Geometry check sheet. Reference: the model listing, model coordinates, mm. Face numbers are marked on the shaded views. A direction names the side the tool comes from. Coordinates: 2 decimals unless noted, no trailing zeros. Loops run counter-clockwise (first coordinate to the right, second up) from the corner with the lowest first, then second, coordinate; pieces in that order, holes last. Notation, with made-up numbers: (-4, 52.5) -> (7, 52.5) arc R13 cw to (7, 65.5) -> close; hole circle Ø4 at (86, -10). An arc over 180 degrees is marked (long way). Answer as a JSON object with one key per item and string values.
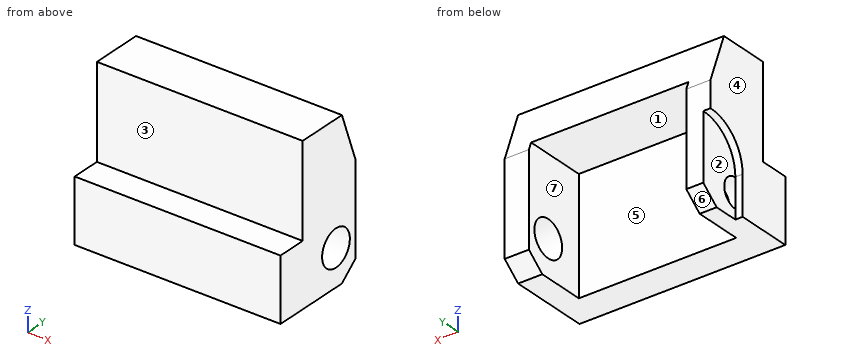
from build123d import *

# Parameters (mm, degrees)
BEARING_BLOCK_DEPTH    = 42.5
LUG_SLOT_PROFILE_W     = 65
LUG_SLOT_PROFILE_H     = 50
LUG_SLOT_65X50_DEPTH   = 27
BORE_15_SKETCH_R       = 7.5
PIVOT_BORE_15_DEPTH    = 10
LUG_RECESS_A_3MM_DEPTH = 3
LUG_RECESS_B_3MM_DEPTH = 3
BORE_10_SKETCH_R       = 6
PIVOT_BORE_10_DEPTH    = 7


with BuildPart() as part:
    # Bearing Block Profile → Bearing Block (new, symmetric)
    with BuildSketch(Plane(origin=(0, 0, 0), x_dir=(0, 0, -1), z_dir=(1, 0, 0))):
        Polygon((0, 0), (38, 0), (38, -12), (64, -12), (64, 21.206684422), (58, 28.458711219), (20, 28.458711219), (0, 21.206684422), align=None)
    extrude(amount=BEARING_BLOCK_DEPTH, both=True)

    # Lug Slot Profile → Lug Slot 65x50 (cut)
    with BuildSketch(Plane(origin=(0, 28.458711219, 0), x_dir=(1, 0, 0), z_dir=(0, 1, 0))):
        with Locations((0, 41.768401258)):
            Rectangle(LUG_SLOT_PROFILE_W, LUG_SLOT_PROFILE_H)
    extrude(amount=-LUG_SLOT_65X50_DEPTH, mode=Mode.SUBTRACT)

    # Bore Ø15 Sketch → Pivot Bore Ø15 (cut)
    with BuildSketch(Plane(origin=(42.5, 0, 0), x_dir=(0, 0, -1), z_dir=(1, 0, 0))):
        with Locations((49, 18)):
            Circle(BORE_15_SKETCH_R)
    extrude(amount=-PIVOT_BORE_15_DEPTH, mode=Mode.SUBTRACT)

    # Lug Recess A Profile → Lug Recess A 3mm (cut)
    with BuildSketch(Plane.ZY.offset(42.5)):
        with BuildLine():
            Line((-58, 28.458711219), (-63.551815655, 21.748391902))
            ThreePointArc((-63.551815655, 21.748391902), (-44.368906721, 11.436763576), (-30.783363951, 28.458711219))
            Line((-30.783363951, 28.458711219), (-58, 28.458711219))
        make_face()
    extrude(amount=-LUG_RECESS_A_3MM_DEPTH, mode=Mode.SUBTRACT)

    # Lug Recess B Profile → Lug Recess B 3mm (cut)
    with BuildSketch(Plane.ZY.offset(42.5)):
        Polygon((-47.779389931, 11.091150514), (-64, 11.091150514), (-64, 21.206684422), (-63.551815655, 21.748391902), align=None)
    extrude(amount=-LUG_RECESS_B_3MM_DEPTH, mode=Mode.SUBTRACT)

    # Bore Ø10 Sketch → Pivot Bore Ø10 (cut)
    with BuildSketch(Plane.ZY.offset(39.5)):
        with Locations(Location((-54, 11.091150514, 0), (0, 0, 180))):
            Circle(BORE_10_SKETCH_R)
    extrude(amount=-PIVOT_BORE_10_DEPTH, mode=Mode.SUBTRACT)


solid = part.part
1. Mould release check, pull along X, two halves, no side actions. Record for the marked faces 4, 5, 6 and 7: released by +X, released by -X, zero draft, split by the parting line, or undercut.
Evaluation:
{"face 4": "released by -X", "face 5": "undercut", "face 6": "zero draft", "face 7": "undercut"}
2. Tool access check on the marked faces 1, 2 and 3. Record the directions out of +Z, -Z, +X, -X, +Y, -Y that give a thin tool (end or side, any length) a straight path to the whole face; none if there is none.
Evaluation:
{"face 1": "-Z, +Y", "face 2": "-Z, -X, +Y", "face 3": "+Z, +X, -X, -Y"}
3. Depth check by flat-ended pin: P1, Ø1.5, axis at x = -17.5, z = -27, coming from the -Y side; P2, Ø10, axis at x = 31.5, z = -19.5, coming from the +Y side; P3, Ø6, axis at x = -10, y = -5, coming from the +Z side; P4, Ø0.9, axis at x = -41, z = -53, coming from the +Y side. Enter the tip coordinate at first touch or a pass-through.
Evaluation:
{"P1": "stops at y = 0", "P2": "stops at y = 28.46", "P3": "stops at z = -38", "P4": "stops at y = 11.09"}
4. Section check B-B, the plane z = -49. Record the boundary of the cut face in (x, y).
Evaluation:
{"outline": "(-42.5, -12) -> (42.5, -12) -> (42.5, 10.5) -> (32.5, 10.5) -> (32.5, 1.46) -> (-32.5, 1.46) -> (-32.5, 7.77) -> (-39.5, 7.77) -> (-39.5, 11.09) -> (-42.5, 11.09) -> close; (-39.5, 14.41) -> (-32.5, 14.41) -> (-32.5, 28.46) -> (-39.5, 28.46) -> close; (32.5, 25.5) -> (42.5, 25.5) -> (42.5, 28.46) -> (32.5, 28.46) -> close"}
5. Section check A-A, the plane y = 3. Record the boundary of the cut face in (x, z).
Evaluation:
{"outline": "(-42.5, -64) -> (-32.5, -64) -> (-32.5, -16.77) -> (32.5, -16.77) -> (32.5, -64) -> (42.5, -64) -> (42.5, 0) -> (-42.5, 0) -> close"}
6. Thickness scan on probe 1 along Y at (x, z) = (37, -49); probe 2 along Y at (x, z) = (-34, -54); probe 3 along X at (y, z) = (12, -42). Record the ranges inside material, lowest first. Write a range as from..to.
Evaluation:
{"probe 1": "y = -12..10.5, 25.5..28.46", "probe 2": "y = -12..5.09, 17.09..28.46", "probe 3": "x = -42.5..-32.5, 32.5..42.5"}
7. Section check D-D, the plane x = -27.5. Record the boundary of the cut face in (y, z).
Evaluation:
{"outline": "(-12, -64) -> (1.46, -64) -> (1.46, -16.77) -> (27.29, -16.77) -> (21.21, 0) -> (0, 0) -> (0, -38) -> (-12, -38) -> close"}
8. Section check C-C, the plane y = 13. Record the boundary of the cut face in (x, z), then the cut area to 3 significant figures.
Evaluation:
{"outline": "(-42.5, -39.95) -> (-39.5, -39.95) -> (-39.5, -48.31) -> (-32.5, -48.31) -> (-32.5, -16.77) -> (32.5, -16.77) -> (32.5, -43.41) -> (42.5, -43.41) -> (42.5, 0) -> (-42.5, 0) -> close; (-39.5, -64) -> (-32.5, -64) -> (-32.5, -59.69) -> (-39.5, -59.69) -> close; (32.5, -64) -> (42.5, -64) -> (42.5, -54.59) -> (32.5, -54.59) -> close", "area": "2,110 mm^2"}
